from build123d import *

# Parameters (mm, degrees)
SKETCH1_W             = 60
SKETCH1_H             = 75
BOSS_EXTRUDE1_DEPTH   = 10
M5_TAPPED_HOLE1_D     = 4.2
M5_TAPPED_HOLE1_DEPTH = 12.4
M5_TAPPED_HOLE1_TIP   = 1.2618073
M5_TAPPED_HOLE2_D     = 4.2
M5_TAPPED_HOLE2_DEPTH = 12.4
M5_TAPPED_HOLE2_TIP   = 1.2618073
SKETCH9_W             = 25
SKETCH9_H             = 40
CUT_EXTRUDE1_DEPTH    = 97.566039579
FILLET1_R             = 5
CHAMFER1_SIZE         = 2


with BuildPart() as part:
    # Sketch1 → Boss-Extrude1 (new body)
    with BuildSketch(Plane(origin=(0, 0, 0), x_dir=(1, 0, 0), z_dir=(0, 1, 0))):
        with Locations((30, 37.5)):
            Rectangle(SKETCH1_W, SKETCH1_H)
    extrude(amount=BOSS_EXTRUDE1_DEPTH)

    # M5 Tapped Hole1
    with Locations(Plane(origin=(0, 0, -75), x_dir=(-1, 0, 0), z_dir=(0, 0, -1))):
        with Locations((-7.5, 5), (-52.5, 5)):
            Hole(M5_TAPPED_HOLE1_D / 2, depth=M5_TAPPED_HOLE1_DEPTH)
            with Locations((0, 0, -(M5_TAPPED_HOLE1_DEPTH + M5_TAPPED_HOLE1_TIP / 2))):  # 118° drill point
                Cone(0, M5_TAPPED_HOLE1_D / 2, M5_TAPPED_HOLE1_TIP, mode=Mode.SUBTRACT)

    # M5 Tapped Hole2
    with Locations(Plane.XY):
        with Locations((52.5, 5), (7.5, 5)):
            Hole(M5_TAPPED_HOLE2_D / 2, depth=M5_TAPPED_HOLE2_DEPTH)
            with Locations((0, 0, -(M5_TAPPED_HOLE2_DEPTH + M5_TAPPED_HOLE2_TIP / 2))):  # 118° drill point
                Cone(0, M5_TAPPED_HOLE2_D / 2, M5_TAPPED_HOLE2_TIP, mode=Mode.SUBTRACT)

    # Sketch9 → Cut-Extrude1 (cut, through all)
    with BuildSketch(Plane(origin=(0, 10, 0), x_dir=(1, 0, 0), z_dir=(0, 1, 0))):
        with Locations((47.5, 37.5)):
            Rectangle(SKETCH9_W, SKETCH9_H)
    extrude(amount=-CUT_EXTRUDE1_DEPTH, mode=Mode.SUBTRACT)

    # Fillet1
    fillet1_edges = [part.edges().sort_by_distance(p)[0] for p in [
        (35, 5, -17.5),
        (35, 5, -57.5),
        (60, 5, -57.5),
        (60, 5, -17.5),
    ]]
    fillet(fillet1_edges, radius=FILLET1_R)

    # Chamfer1
    chamfer1_edges = [part.edges().sort_by_distance(p)[0] for p in [
        (60, 10, -6.25),
        (47.5, 10, -57.5),
        (47.5, 0, -57.5),
        (35, 10, -37.5),
        (60, 10, -68.75),
        (60, 0, -6.25),
        (47.5, 10, -17.5),
        (58.535533906, 10, -16.035533906),
        (58.535533906, 10, -58.964466094),
        (60, 0, -68.75),
        (35, 0, -37.5),
        (47.5, 0, -17.5),
        (58.535533906, 0, -16.035533906),
        (58.535533906, 0, -58.964466094),
        (36.464466094, 10, -18.964466094),
        (36.464466094, 0, -18.964466094),
        (36.464466094, 10, -56.035533906),
        (36.464466094, 0, -56.035533906),
    ]]
    chamfer(chamfer1_edges, length=CHAMFER1_SIZE)


solid = part.part
Work out the finished part from the listing and answer in its coordinate system (mm). A direction names the side the tool comes from. Coordinates: 2 decimals unless noted, no trailing zeros. Write each loop counter-clockwise with the first axis right and the second up, starting at its lowest first coordinate (ties: lowest second). Pieces come first, ordered by that corner, then holes. Notation, with made-up numbers: M 71,26 L 81,26 A16 cw 81,37 Z; hole C 20,72.25 d3. An arc over 180 degrees is marked long. Answer as CSV lines item,"result". Start each with the question number.
Item 1: Section A-A on x = 49 is taken. Write down the section's boundary in (y, z).
Item 2: A tool of negligible diameter and unlimited length cuts with its end or side. For faces 1 (the face through (50.497, 5.631, -6.287)), 2 (the face through (54.503, 5.631, -68.713)), 3 (the face through (35.88, 1.236, -56.531)), 4 (the face through (35.9, 8.8, -56.6)), from which of +Z, -Z, +X, -X, +Y, -Y can it reach the whole face along a straight path? Write none if from no direction.
Item 3: Flat-ended cylindrical pins translate along their axes: P1, Ø3.5, axis at x = 52.5, y = 5, coming from the +Z side; P2, Ø5, axis at y = 5.5, z = -42.5, coming from the +X side. Find the tip coordinate at first contact, or state that the pin passes through.
Item 4: Section B-B on z = -27.5 is taken. Write down the section's boundary in (x, y).
Item 5: Determine the mould class of faces 5 (the face through (57.65, 0.79, -59.79)), 6 (the face through (57.69, 9.24, -15.13)), 7 (the face through (58.57, 4.96, -59)), 8 (the face through (9.048, 6.419, -6.287)) for opening direction Y: released by +Y, released by -Y, zero draft, split by the parting line, or undercut.
Item 6: Consider L1, parallel to X at y = 5, z = -8.25; L2, parallel to Z at x = 51, y = 3.75; L3, parallel to Y at x = 52.5, z = -65.5. Determine where each line is inside the solid, lowest interval first.
Checks:
1,outline,"M 0,-75 L 10,-75 L 10,-59.5 L 8,-57.5 L 2,-57.5 L 0,-59.5 Z; M 0,-15.5 L 2,-17.5 L 8,-17.5 L 10,-15.5 L 10,0 L 0,0 Z"
2,face 1,"+Z"
2,face 2,"-Z"
2,face 3,"+X, -Y"
2,face 4,"+X, +Y"
3,P1,"stops at z = -12.61"
3,P2,"stops at x = 35"
4,outline,"M 0,0 L 33,0 L 35,2 L 35,8 L 33,10 L 0,10 Z"
5,face 5,"released by -Y"
5,face 6,"released by +Y"
5,face 7,"zero draft"
5,face 8,"undercut"
6,L1,"x = 0 to 5.4, 9.6 to 50.4, 54.6 to 60"
6,L2,"z = -62.51 to -57.5, -17.5 to -12.49"
6,L3,"y = 0 to 2.9, 7.1 to 10"
